```python
from build123d import *

# Parameters (mm, degrees)
SKETCH_1_R          = 21.75
SKETCH_1_R_2        = 7.5
EXTRUDE_1_DEPTH     = 12
CUT_EXTRUDE_1_DEPTH = 8
SKETCH_4_R          = 21.75
SKETCH_5_R          = 13
SKETCH_6_R          = 6.5
CUT_EXTRUDE_3_DEPTH = 48


with BuildPart() as part:
    # 草图1 → 凸台-拉伸1 (new body)
    with BuildSketch(Plane.XY):
        Circle(SKETCH_1_R)
        Circle(SKETCH_1_R_2, mode=Mode.SUBTRACT)
    extrude(amount=EXTRUDE_1_DEPTH)

    # 草图2 → 切除-拉伸1 (cut)
    with BuildSketch(Plane.XY.offset(12)):
        with BuildLine():
            Line((-11, 3), (11, 3))
            ThreePointArc((11, 3), (11.353553391, 2.853553391), (11.5, 2.5))
            Line((11.5, 2.5), (11.5, -2.5))
            ThreePointArc((11.5, -2.5), (11.353553391, -2.853553391), (11, -3))
            Line((11, -3), (-11, -3))
            ThreePointArc((-11, -3), (-11.353553391, -2.853553391), (-11.5, -2.5))
            Line((-11.5, -2.5), (-11.5, 2.5))
            ThreePointArc((-11.5, 2.5), (-11.353553391, 2.853553391), (-11, 3))
        make_face()
    extrude(amount=-CUT_EXTRUDE_1_DEPTH, mode=Mode.SUBTRACT)

    # 草图4 → 放样2 section 0
    with BuildSketch(Plane(origin=(0, 0, 0), x_dir=(-1, 0, 0), z_dir=(0, 0, -1))):
        Circle(SKETCH_4_R)
    # 草图5 → 放样2 section 1
    with BuildSketch(Plane(origin=(0, 0, -8), x_dir=(-1, 0, 0), z_dir=(0, 0, -1))):
        Circle(SKETCH_5_R)
    loft()

    # 草图6 → 切除-拉伸3 (cut)
    with BuildSketch(Plane.XY):
        Circle(SKETCH_6_R)
    extrude(amount=-CUT_EXTRUDE_3_DEPTH, mode=Mode.SUBTRACT)


solid = part.part
```
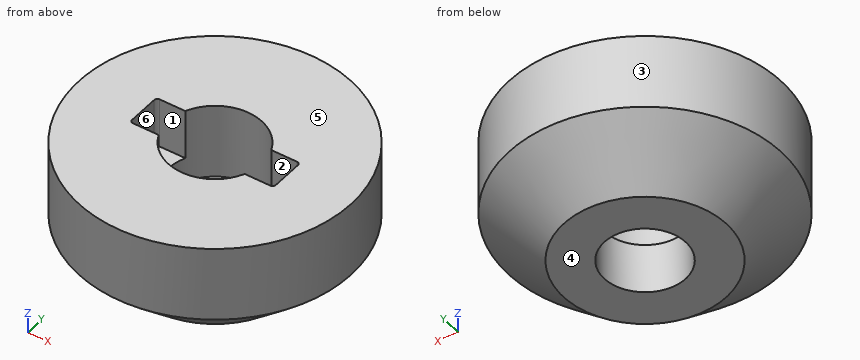
Here's how the part is built. I have some questions about the finished solid (model axes, mm). Face numbers are marked on the shaded views. A direction names the side the tool comes from. Give positions to 0.01 mm unless a question says otherwise; leave off trailing zeros. Write each loop counter-clockwise with the first axis right and the second up, starting at its lowest first coordinate (ties: lowest second). Pieces come first, ordered by that corner, then holes. Notation, with made-up numbers: M 76,-24.5 L 132,-24.5 A32 cw 132,13.5 Z; hole C -30,31 d8. An arc over 180 degrees is marked long. Put each result on its own line as item: value. Start each with the question number.
Item 1: On a 3-axis mill with a long thin cutter (end or side, diameter ignored), from which of +Z, -Z, +X, -X, +Y, -Y can I reach the whole of each face in a straight line? I mean the marked faces 5 and 6. Say none if no direction works.
Item 2: If we section it at B-B, the plane z = 2.5: Write out the boundary of the cut face in (x, y).
Item 3: If we section it at A-A, the plane x = 0: Write out the boundary of the cut face in (y, z).
Item 4: Thinking about a two-plate mould opening in Y: for the marked faces 1, 2, 3 and 4, which applies, +Y half, -Y half, draft (parallel to the pull), parting line (faces both ways), or undercut?
Item 5: I need wall thicknesses on L1, parallel to Y at x = 0, z = 9.75; L2, parallel to Y at x = 0, z = -6; L3, parallel to Z at x = 13.5, y = 9. Which ranges of each line are inside material? Lowest first, please. Write a range as from..to.
Item 6: If we section it at C-C, the plane z = -5.5: Write out the boundary of the cut face in (x, y).
Item 7: Will these pins go through, and if not, where does the flat tip stop? pin 1 (4.5 mm diameter, centred on x = -9, z = 9, fed in from -Y); pin 2 (2 mm diameter, centred on y = -5.5, z = 8, fed in from -X); pin 3 (12 mm diameter, centred on x = 8, z = 4.5, fed in from +Y).
Values:
1. face 5: +Z, +X, -X, +Y, -Y
1. face 6: +Z
2. outline: C 0,0 d43.5; hole C 0,0 d15
3. outline: M -21.75,0 L -13,-8 L -6.5,-8 L -6.5,0 L -7.5,0 L -7.5,12 L -21.75,12 Z; M 6.5,-8 L 13,-8 L 21.75,0 L 21.75,12 L 7.5,12 L 7.5,0 L 6.5,0 Z
4. face 1: undercut
4. face 2: undercut
4. face 3: parting line
4. face 4: draft
5. L1: -21.75..-7.5, 7.5..21.75
5. L2: -15.19..-6.5, 6.5..15.19
5. L3: -5.05..12
6. outline: C 0,0 d31.47; hole C 0,0 d13
7. pin 1: y = -20.68
7. pin 2: x = -21.28
7. pin 3: y = 21.66
